Check sheet for the modelled part. Datum: model origin and axes. Units: mm. A direction names the side the tool comes from. Give positions to 0.01 mm unless a question says otherwise; leave off trailing zeros. Loops run counter-clockwise (first coordinate to the right, second up) from the corner with the lowest first, then second, coordinate; pieces in that order, holes last. Notation, with made-up numbers: (61, 63.5) - (89, 63.5) arc R27 ccw to (89, 102.5) - close; hole circle Ø6 at (-17, -24.75). An arc over 180 degrees is marked (long way). Answer in a Markdown table with one row per item. Add a question column.
(1) Sectioned sample at A-A on z = 5. Enter the section's corners in (x, y).
(2) Sectioned sample at B-B on y = 0. Enter the section's corners in (x, z).
(3) Sectioned sample at C-C on x = -10. Enter the section's corners in (y, z).
(4) Go/stop test with flat-tipped pins: P1, Ø5, axis at y = 7, z = 1, coming from the +X side; P2, Ø4, axis at x = -2.5, z = -0.5, coming from the -Y side; P3, Ø4, axis at x = -13, y = 6, coming from the +Z side. Record where each tip stops, or that it passes through.
(5) Draft check along Z on faces 1 (the face through (0, 5, 3.5)), 2 (the face through (0, 18, 1.5)), 3 (the face through (-4.336, -19.524, -2.486)). Enter one of: released by +Z, released by -Z, zero draft, split by the parting line, or undercut.
(6) Sectioned sample at D-D on x = 6.5. Enter the section's corners in (y, z).
(7) Thickness scan on L1, parallel to Z at x = 10.5, y = 15; L2, parallel to Z at x = -4, y = 11; L3, parallel to Y at x = -10, z = 0.75. Record the ranges inside material, lowest first.
(8) Set-up check for faces 4 (the face through (0, 18, -1.5)), 5 (the face through (-4.336, -19.524, 2.514)), 6 (the face through (-12.827, -6.948, 5.965)), 7 (the face through (6.99, 1.6, 5.96)): record each of +Z, -Z, +X, -X, +Y, -Y from which the full face is reachable in a straight line by a thin tool's end or side.
from build123d import *

# Parameters (mm, degrees)
DISC_PROFILE_40_R      = 20
DISC_40X7_DEPTH        = 3.5
RIM_GROOVE_PROFILE_W   = 3
RIM_GROOVE_PROFILE_H   = 2.5
THROUGH_HOLE_PROFILE_R = 2.5
THROUGH_HOLE_DEPTH     = 47
U_HOOK_BOSS_DEPTH      = 5


with BuildPart() as part:
    # Disc Profile Ø40 → Disc Ø40x7 (new, symmetric)
    with BuildSketch(Plane.XY):
        Circle(DISC_PROFILE_40_R)
    extrude(amount=DISC_40X7_DEPTH, both=True)

    # Rim Groove Profile → Rim Groove (revolve, cut)
    with BuildSketch(Plane(origin=(0, 0, 0), x_dir=(0, 0, -1), z_dir=(1, 0, 0)), mode=Mode.PRIVATE) as rim_groove_sk:
        with Locations((0, 18.75)):
            Rectangle(RIM_GROOVE_PROFILE_W, RIM_GROOVE_PROFILE_H)
    revolve(rim_groove_sk.sketch.rotate(Axis((0, 0, 14.756637323), (0, 0, -1)), 90), axis=Axis((0, 0, 14.756637323), (0, 0, -1)), mode=Mode.SUBTRACT)

    # Through Hole Profile → Through Hole (cut)
    with BuildSketch(Plane.XY.offset(3.5)):
        with Locations((-10, 0)):
            Circle(THROUGH_HOLE_PROFILE_R)
    extrude(amount=-THROUGH_HOLE_DEPTH, mode=Mode.SUBTRACT)

    # U Hook Profile → U Hook Boss (add)
    with BuildSketch(Plane.XY.offset(3.5)):
        with BuildLine():
            Line((-19.259231956, 1.231512725), (-2.70246973, -5.830613343))
            Line((-2.70246973, -5.830613343), (5.144337012, 12.56578913))
            Line((5.144337012, 12.56578913), (10.663257754, 10.211747107))
            Line((10.663257754, 10.211747107), (3.208791349, -7.264835242))
            ThreePointArc((3.208791349, -7.264835242), (-0.072222189, -10.477818578), (-4.664171415, -10.429713961))
            Line((-4.664171415, -10.429713961), (-21.220933641, -3.367587893))
            ThreePointArc((-21.220933641, -3.367587893), (-24.433916977, -0.086574356), (-24.38581236, 4.505374871))
            Line((-24.38581236, 4.505374871), (-16.931345956, 21.981957221))
            Line((-16.931345956, 21.981957221), (-11.412425214, 19.627915198))
            Line((-11.412425214, 19.627915198), (-19.259231956, 1.231512725))
        make_face()
    extrude(amount=U_HOOK_BOSS_DEPTH)


solid = part.part
Reply:
| question | item | result |
|---|---|---|
| 1 | outline | (-24.39, 4.51) arc R6 ccw to (-21.22, -3.37) - (-4.66, -10.43) arc R6 ccw to (3.21, -7.26) - (10.66, 10.21) - (5.14, 12.57) - (-2.7, -5.83) - (-19.26, 1.23) - (-11.41, 19.63) - (-16.93, 21.98) - close |
| 2 | outline | (-24.47, 3.5) - (-20, 3.5) - (-20, 1.5) - (-17.5, 1.5) - (-17.5, -1.5) - (-20, -1.5) - (-20, -3.5) - (-12.5, -3.5) - (-12.5, 3.5) - (-16.37, 3.5) - (-16.37, 8.5) - (-24.47, 8.5) - close; (-7.5, -3.5) - (20, -3.5) - (20, -1.5) - (17.5, -1.5) - (17.5, 1.5) - (20, 1.5) - (20, 3.5) - (6.31, 3.5) - (6.31, 8.5) - (-0.22, 8.5) - (-0.22, 3.5) - (-7.5, 3.5) - close |
| 3 | outline | (-17.32, -3.5) - (-2.5, -3.5) - (-2.5, 3.5) - (-2.72, 3.5) - (-2.72, 8.5) - (-8.15, 8.5) - (-8.15, 3.5) - (-17.32, 3.5) - (-17.32, 1.5) - (-14.36, 1.5) - (-14.36, -1.5) - (-17.32, -1.5) - close; (2.5, -3.5) - (17.32, -3.5) - (17.32, -1.5) - (14.36, -1.5) - (14.36, 1.5) - (17.32, 1.5) - (17.32, 3.5) - (2.5, 3.5) - close |
| 4 | P1 | x = 19.48 |
| 4 | P2 | y = -19.99 |
| 4 | P3 | z = 3.5 |
| 5 | face 1 | released by +Z |
| 5 | face 2 | undercut |
| 5 | face 3 | zero draft |
| 6 | outline | (-18.91, -3.5) - (18.91, -3.5) - (18.91, -1.5) - (16.25, -1.5) - (16.25, 1.5) - (18.91, 1.5) - (18.91, 3.5) - (11.99, 3.5) - (11.99, 8.5) - (0.45, 8.5) - (0.45, 3.5) - (-18.91, 3.5) - (-18.91, 1.5) - (-16.25, 1.5) - (-16.25, -1.5) - (-18.91, -1.5) - close |
| 7 | L1 | -3.5 to -1.5, 1.5 to 3.5 |
| 7 | L2 | -3.5 to 3.5 |
| 7 | L3 | -14.36 to -2.5, 2.5 to 14.36 |
| 8 | face 4 | none |
| 8 | face 5 | -Z |
| 8 | face 6 | +Z, -X, -Y |
| 8 | face 7 | +Z, +X, -Y |
